The model under review builds one solid part; all positions refer to its coordinate system, in mm. A direction names the side the tool comes from. Round coordinates to 2 decimals unless told otherwise and drop trailing zeros. Loops run counter-clockwise (first coordinate to the right, second up) from the corner with the lowest first, then second, coordinate; pieces in that order, holes last. Notation, with made-up numbers: M -7,-1.5 L 30,-1.5 A13 ccw 30,8.5 Z; hole C 41,-28 d10. An arc over 180 degrees is marked long. Answer as a JSON object with one key per item and string values. Group by question number.
Item 1: To check wall thickness, follow line 1 (Y direction, x = 244.5, z = 9); line 2 (X direction, y = -608.5, z = 0); line 3 (Y direction, x = 269, z = 13). State the ranges of each line that lie inside material, in increasing order.
Item 2: Consider section C-C (y = -596.5). Give the boundary of the cut face in (x, z).
Item 3: Consider section B-B (y = -572.5). Give the boundary of the cut face in (x, z).
Item 4: Tool access review of faces 3 (the face through (229.484, -607.796, -2.604)), 4 (the face through (224.527, -602.274, -3.255)), 5 (the face through (267.3, -600, 9.2)): name each direction out of +Z, -Z, +X, -X, +Y, -Y from which nothing blocks a thin tool from reaching the whole face with its end or side.
Item 5: Consider section A-A (z = 0). Give the boundary of the cut face in (x, y).
Item 6: The part is to be moulded in two halves that separate along Z. For faces 1 (the face through (258.1, -581.44, -1.95)), 2 (the face through (249, -567, 0)), say which applies: +Z half, -Z half, draft (parallel to the pull), parting line (faces both ways), or undercut.
Item 7: Insertion check: P1, Ø2, axis at y = -590, z = 8, coming from the -X side; P2, Ø1, axis at y = -602, z = 8.5, coming from the -X side; P3, Ø10, axis at y = -577.5, z = -5, coming from the -X side. Each pin has a flat end and moves straight along its axis. Give the tip position at first contact, or say it passes through.
```python
from build123d import *

# Parameters (mm, degrees)
CHAMFER1_SIZE = 0.5


with BuildPart() as part:
    # Sketch1 → Revolve1 (revolve)
    with BuildSketch(Plane.XY, mode=Mode.PRIVATE) as revolve1_sk:
        Polygon((258.314300847, -567), (258.314300847, -595), (269.314300847, -595), (269.314300847, -600), (274.314300847, -600), (274.314300847, -604.5), (269.314300847, -604.5), (269.314300847, -611.5), (249.314300847, -611.5), (249.314300847, -567), align=None)
    revolve(revolve1_sk.sketch.rotate(Axis((249.314300847, -567, 0), (0, -1, 0)), 90), axis=Axis((249.314300847, -567, 0), (0, -1, 0)))

    # Chamfer1
    chamfer1_edges = [part.edges().sort_by_distance(p)[0] for p in [
        (249.314300847, -604.5, -25),
        (249.314300847, -611.5, -20),
        (249.314300847, -567, -9),
        (249.314300847, -595, -20),
        (249.314300847, -600, -25),
    ]]
    chamfer(chamfer1_edges, length=CHAMFER1_SIZE)


solid = part.part
```
Geometry results:
{
 "1": {"line 1": "y = -611.5 to -595", "line 2": "x = 229.31 to 269.31", "line 3": "y = -604.5 to -600"},
 "2": {"outline": "C 249.31,0 d40"},
 "3": {"outline": "C 249.31,0 d18"},
 "4": {"face 3": "-Y", "face 4": "+Y, -Y", "face 5": "+Y"},
 "5": {"outline": "M 224.31,-604 L 224.81,-604.5 L 229.31,-604.5 L 229.31,-611 L 229.81,-611.5 L 268.81,-611.5 L 269.31,-611 L 269.31,-604.5 L 273.81,-604.5 L 274.31,-604 L 274.31,-600.5 L 273.81,-600 L 269.31,-600 L 269.31,-595.5 L 268.81,-595 L 258.31,-595 L 258.31,-567.5 L 257.81,-567 L 240.81,-567 L 240.31,-567.5 L 240.31,-595 L 229.81,-595 L 229.31,-595.5 L 229.31,-600 L 224.81,-600 L 224.31,-600.5 Z"},
 "6": {"face 1": "parting line", "face 2": "draft"},
 "7": {"P1": "stops at x = 243.66", "P2": "stops at x = 225.63", "P3": "stops at x = 240.31"}
}
